Input: part model. Units: mm. Frame: model coordinates. A direction names the side the tool comes from. Coordinates: 2 decimals unless noted, no trailing zeros. Write each loop counter-clockwise with the first axis right and the second up, starting at its lowest first coordinate (ties: lowest second). Pieces come first, ordered by that corner, then holes. Notation, with made-up numbers: (39.25, 34) - (60.25, 34) arc R9 ccw to (60.25, 49) - close; hole circle Ø7 at (19, 12). An arc over 180 degrees is marked (long way). Use a Markdown table: item, result. Add a question column.
Q1. Section query C-C (z = -60). Return the cut outline in (x, y), then the cut area to 3 significant figures.
Q2. Mould query, pull axis X, two halves, no side actions, for faces 1 (the face through (-51, 0, -46)), 2 (the face through (41.293, -0.042, -3.909)), 3 (the face through (49, 3, -109)). Classes: released by +X, released by -X, zero draft, split by the parting line, or undercut.
Q3. Set-up query: faces 4 (the face through (-33, 0, -24.5)), 5 (the face through (-29, 0, -68)), 6 (the face through (49, -3, -109)), 7 (the face through (-9, 0, -56)), 8 (the face through (60.97, 5.48, -136.14)). Return all of +Z, -Z, +X, -X, +Y, -Y with unobstructed straight access to the full face (end or side cutting, diameter ignored); none if empty.
Q4. Pin query (flat end, axial travel): P1, Ø5, axis at x = -86, z = -49, coming from the +Y side; P2, Ø9, axis at x = 52, z = -108.5, coming from the -Y side; P3, Ø4.5, axis at y = -0.5, z = -51, coming from the +X side; P4, Ø9, axis at x = 32, z = -13, coming from the -Y side. Return the tip coordinate at first contact, or that it passes through.
Q5. Section query B-B (y = 0). Give the number of separate pieces and of enclosed holes in the cut face, then the cut area to 3 significant figures.
Q6. Material intervals for probe 1 along X at (y, z) = (-1.3, -13); probe 2 along X at (y, z) = (3.5, -99); probe 3 along X at (y, z) = (4.5, -8.5), sorted ascending. Write a range as from..to.
Q7. Section query A-A (z = -34). Return the cut outline in (x, y).
Q8. Section query D-D (x = 43). Return the cut outline in (y, z), then the cut area to 3 significant figures.
from build123d import *
from build123d.topology import SkipClean

# Parameters (mm, degrees)
BASE_PLATE_SKETCH_W              = 9
BASE_PLATE_SKETCH_H              = 30
BASE_PLATE_DEPTH                 = 7.5
RAISED_PAD_SKETCH_R              = 5.5
RAISED_PAD_DEPTH                 = 3
ARM_BLOCK_SKETCH_R               = 5
ARM_BLOCK_DEPTH                  = 9
FIRST_START                      = 31.5
FIRST_ARM_PIVOT_BOSS_SKETCH_R    = 9
FIRST_ARM_PIVOT_BOSS_SKETCH_R_2  = 5
FIRST_ARM_PIVOT_BOSS_DEPTH       = 31.5
ARM_RIB_REACH                    = 177.026
ARM_RIB_SKETCH_WALL_W            = 384.00451541
ARM_RIB_SKETCH_WALL_H            = 6
SECOND_START                     = -9
SECOND_ARM_DEPTH                 = 9
SECOND_ARM_PIVOT_BOSS_DEPTH      = 11
SECOND_ARM_PIVOT_BOSS_DEPTH_BACK = 19
SECOND_ARM_PIVOT_BOSS_SKETCH_R   = 12
PIVOT_BORE_SKETCH_R              = 5
PIVOT_BORE_DEPTH                 = 214.225819262


with BuildPart() as part:
    # Base Plate Sketch → Base Plate (new, symmetric)
    with BuildSketch(Plane(origin=(0, 0, 0), x_dir=(1, 0, 0), z_dir=(0, 1, 0))):
        with BuildLine():
            Line((-43, 24.5), (-23, 24.5))
            ThreePointArc((-23, 24.5), (-20.878679656, 23.621320344), (-20, 21.5))
            Line((-20, 21.5), (-20, 0))
            Line((-20, 0), (0, 0))
            Line((0, 0), (0, 90))
            Line((0, 90), (-22, 90))
            Line((-22, 90), (-36, 46))
            Line((-36, 46), (-66, 46))
            Line((-66, 46), (-66, 0))
            Line((-66, 0), (-46, 0))
            Line((-46, 0), (-46, 21.5))
            ThreePointArc((-46, 21.5), (-45.121320344, 23.621320344), (-43, 24.5))
        make_face()
        with Locations((-13.5, 56)):
            Rectangle(BASE_PLATE_SKETCH_W, BASE_PLATE_SKETCH_H, mode=Mode.SUBTRACT)
    extrude(amount=BASE_PLATE_DEPTH, both=True)

    # Raised Pad Sketch → Raised Pad (add, symmetric)
    # profile 1 of 2: a face of its own
    with BuildSketch(Plane(origin=(0, 0, 0), x_dir=(1, 0, 0), z_dir=(0, 1, 0))):
        with BuildLine():
            Line((0, 82), (45, 82))
            Line((45, 82), (45, 13))
            ThreePointArc((45, 13), (41.192388155, 3.807611845), (32, 0))
            Line((32, 0), (0, 0))
            Line((0, 0), (0, 82))
        make_face()
        with Locations(Location((32, 13, 0), (0, 0, 270))):
            Circle(RAISED_PAD_SKETCH_R, mode=Mode.SUBTRACT)
    # profile 2 of 2: a face of its own
    with BuildSketch(Plane(origin=(0, 0, 0), x_dir=(1, 0, 0), z_dir=(0, 1, 0))):
        with BuildLine():
            Line((-66, 0), (-90, 0))
            ThreePointArc((-90, 0), (-99.192388155, 3.807611845), (-103, 13))
            Line((-103, 13), (-103, 130))
            Line((-103, 130), (-83, 130))
            Line((-83, 130), (-83, 98))
            Line((-83, 98), (-66, 46))
            Line((-66, 46), (-66, 0))
        make_face()
        with Locations(Location((-90, 13, 0), (0, 0, 270))):
            Circle(RAISED_PAD_SKETCH_R, mode=Mode.SUBTRACT)
    extrude(amount=RAISED_PAD_DEPTH, both=True)

    # Arm Block Sketch → Arm Block (add)
    with BuildSketch(Plane(origin=(45, 0, 0), x_dir=(0, 0, -1), z_dir=(1, 0, 0))):
        with BuildLine():
            Line((45, 0), (45, 12))
            Line((45, 12), (129, 12))
            ThreePointArc((129, 12), (141, 0), (129, -12))
            Line((129, -12), (45, -12))
            Line((45, -12), (45, 0))
        make_face()
        with Locations((129, 0)):
            Circle(ARM_BLOCK_SKETCH_R, mode=Mode.SUBTRACT)
    extrude(amount=-ARM_BLOCK_DEPTH)

    # First Arm Pivot Boss Sketch → First Arm Pivot Boss (add)
    with BuildSketch(Plane(origin=(45, 0, 0), x_dir=(0, 0, -1), z_dir=(1, 0, 0)).offset(FIRST_START)):
        with Locations(Location((129, 0, 0), (0, 0, 180))):
            Circle(FIRST_ARM_PIVOT_BOSS_SKETCH_R)
        with Locations((129, 0)):
            Circle(FIRST_ARM_PIVOT_BOSS_SKETCH_R_2, mode=Mode.SUBTRACT)
    extrude(amount=-FIRST_ARM_PIVOT_BOSS_DEPTH)

    # Arm Rib Sketch wall → Arm Rib (add, up to next)
    with BuildSketch(Plane(origin=(50.5, 0, -105), x_dir=(0.344254649158, 0, -0.938876315887), z_dir=(-0.938876315887, 0, -0.344254649158)), mode=Mode.PRIVATE) as arm_rib_sk1:
        Rectangle(ARM_RIB_SKETCH_WALL_W, ARM_RIB_SKETCH_WALL_H)
    arm_rib_tool1 = extrude(arm_rib_sk1.sketch, amount=ARM_RIB_REACH, mode=Mode.PRIVATE) - part.part
    add(arm_rib_tool1.solids().sort_by_distance((50.5, 0, -105))[0])

    # Second Arm Sketch → Second Arm (add)
    with BuildSketch(Plane.ZY.offset(103).offset(SECOND_START)):
        with BuildLine():
            Line((-45, 0), (-45, 12))
            Line((-45, 12), (-129, 12))
            ThreePointArc((-129, 12), (-141, 0), (-129, -12))
            Line((-129, -12), (-45, -12))
            Line((-45, -12), (-45, 0))
        make_face()
    extrude(amount=SECOND_ARM_DEPTH)

    # Second Arm Pivot Boss Sketch → Second Arm Pivot Boss (add, two sides: drawn at the far end of the back side and taken through both)
    with SkipClean():  # the faces are left unmerged after this step: merging them gives an invalid solid
        with BuildSketch(Plane(origin=(-94, 0, 0), x_dir=(0, 0, -1), z_dir=(1, 0, 0)).offset(-SECOND_ARM_PIVOT_BOSS_DEPTH_BACK)):
            with Locations(Location((129, 0, 0), (0, 0, 194.477512186))):
                Circle(SECOND_ARM_PIVOT_BOSS_SKETCH_R)
        extrude(amount=SECOND_ARM_PIVOT_BOSS_DEPTH + SECOND_ARM_PIVOT_BOSS_DEPTH_BACK)

    # Pivot Bore Sketch → Pivot Bore (cut, through all)
    with SkipClean():  # the faces are left unmerged after this step: merging them gives an invalid solid
        with BuildSketch(Plane(origin=(-83, 0, 0), x_dir=(0, 0, -1), z_dir=(1, 0, 0))):
            with Locations((129, 0)):
                Circle(PIVOT_BORE_SKETCH_R)
        extrude(amount=-PIVOT_BORE_DEPTH, mode=Mode.SUBTRACT)


solid = part.part
Values follow:
| question | item | result |
|---|---|---|
| 1 | outline | (-103, -12) - (-94, -12) - (-94, -3) - (-70.58, -3) - (-70.58, 3) - (-94, 3) - (-94, 12) - (-103, 12) - close; (-31.55, -7.5) - (-18, -7.5) - (-18, 7.5) - (-31.55, 7.5) - close; (-9, -7.5) - (0, -7.5) - (0, -3) - (36, -3) - (36, -12) - (45, -12) - (45, 12) - (36, 12) - (36, 3) - (0, 3) - (0, 7.5) - (-9, 7.5) - close |
| 1 | area | 1,130 mm2 |
| 2 | face 1 | undercut |
| 2 | face 2 | released by +X |
| 2 | face 3 | zero draft |
| 3 | face 4 | +Z, +Y, -Y |
| 3 | face 5 | -Z, +Y, -Y |
| 3 | face 6 | +Z, +X, -Y |
| 3 | face 7 | +Y, -Y |
| 3 | face 8 | +X |
| 4 | P1 | y = 3 |
| 4 | P2 | y = -3 |
| 4 | P3 | x = 45 |
| 4 | P4 | through |
| 5 | separate pieces | 3 |
| 5 | enclosed holes | 3 |
| 5 | area | 11,700 mm2 |
| 6 | probe 1 | -103..-95.5, -84.5..-46, -20..26.5, 37.5..45 |
| 6 | probe 2 | -103..-94, 36..45 |
| 6 | probe 3 | -66..-46, -20..0 |
| 7 | outline | (-103, -3) - (-66, -3) - (-66, -7.5) - (0, -7.5) - (0, -3) - (45, -3) - (45, 3) - (0, 3) - (0, 7.5) - (-66, 7.5) - (-66, 3) - (-103, 3) - close |
| 8 | outline | (-12, -129) arc R12 ccw to (12, -129) - (12, -45) - (3, -45) - (3, -6.07) - (-3, -6.07) - (-3, -45) - (-12, -45) - close; hole circle Ø10 at (0, -129) |
| 8 | area | 2,400 mm2 |
